Check sheet for the modelled part. Datum: model origin and axes. Units: mm. A direction names the side the tool comes from. Round coordinates to 2 decimals unless told otherwise and drop trailing zeros.
(1) Thickness scan on probe 1 along Z at (x, y) = (-34, 2.1); probe 2 along Z at (x, y) = (-15, 3.3); probe 3 along Z at (x, y) = (21, -2.55). Record the ranges inside material, lowest first.
(2) Tool access check on faces 1 (the flat face through (-1, 0, -230)), 2 (the flat face through (-11, -0.4, -198)), 3 (the flat face through (-12.8, -0.7, -177.8)). Record the directions out of +Z, -Z, +X, -X, +Y, -Y that give a thin tool (end or side, any length) a straight path to the whole face; none if there is none.
(3) Sectioned sample at A-A, the plane y = 2. Count the separate pieces of the cut face and the enclosed holes in it, and give its area (3 significant figures).
(4) Depth check by flat-ended pin: pin 1 (2.5 mm diameter, centred on x = -7.5, z = -199, fed in from -Y); pin 2 (5 mm diameter, centred on x = -14.5, z = -61, fed in from +Y); pin 3 (3.5 mm diameter, centred on x = -34, z = 0, fed in from +Y). Enter the tip coordinate at first touch or a pass-through.
```python
from build123d import *

# Parameters (mm, degrees)
SKETCH_1_W                = 80
SKETCH_1_H                = 10
EXTRUDE_1_DEPTH           = 230
HOLE_WIZARD_1_D           = 4.5
HOLE_WIZARD_1_CBORE_D     = 8
HOLE_WIZARD_1_CBORE_DEPTH = 4.6
HOLE_WIZARD_2_D           = 5.5
HOLE_WIZARD_2_CBORE_D     = 10
HOLE_WIZARD_2_CBORE_DEPTH = 5.7


with BuildPart() as part:
    # 草图1 → 凸台-拉伸1 (new, symmetric)
    with BuildSketch(Plane.XY):
        Rectangle(SKETCH_1_W, SKETCH_1_H)
    extrude(amount=EXTRUDE_1_DEPTH, both=True)

    # 打孔尺寸(%根据)内六角圆柱头螺钉的类型1 (through all)
    with Locations(Plane(origin=(0, -5, 0), x_dir=(-1, 0, 0), z_dir=(0, -1, 0))):
        with Locations((34, -200), (9, -200), (-21, -200), (34, 0), (9, 0), (-21, 0), (34, 200), (9, 200), (-21, 200)):
            CounterBoreHole(HOLE_WIZARD_1_D / 2, HOLE_WIZARD_1_CBORE_D / 2, HOLE_WIZARD_1_CBORE_DEPTH)

    # 打孔尺寸(%根据)内六角圆柱头螺钉的类型2 (through all)
    with Locations(Plane(origin=(0, 5, 0), x_dir=(1, 0, 0), z_dir=(0, 1, 0))):
        with Locations((-15, -180), (25, -180), (-15, -60), (25, -60), (25, 60), (25, 180), (-15, 180), (-15, 60)):
            CounterBoreHole(HOLE_WIZARD_2_D / 2, HOLE_WIZARD_2_CBORE_D / 2, HOLE_WIZARD_2_CBORE_DEPTH)


solid = part.part
```
Derived:
1. probe 1: z = -230 to -202.25, -197.75 to -2.25, 2.25 to 197.75, 202.25 to 230
1. probe 2: z = -230 to -185, -175 to -65, -55 to 55, 65 to 175, 185 to 230
1. probe 3: z = -230 to -204, -196 to -4, 4 to 196, 204 to 230
2. face 1: -Z, +X, -X, +Y, -Y
2. face 2: -Y
2. face 3: +Y
3. separate pieces: 1
3. enclosed holes: 17
3. area: 36,000 mm2
4. pin 1: stops at y = -0.4
4. pin 2: stops at y = -0.7
4. pin 3: passes through
